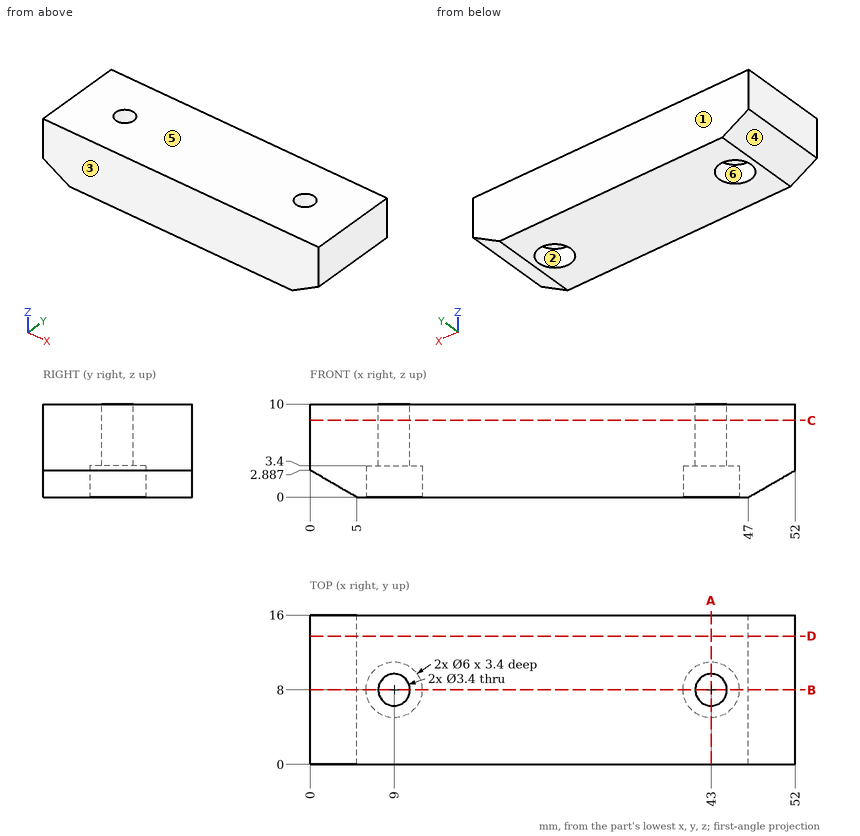
Check sheet for the drawn part. Datum: minimum x, y, z corner. Units: mm. A direction names the side the tool comes from. Give positions to 0.01 mm unless a question says otherwise; leave off trailing zeros. Order: outer loops, then holes, each group sorted by start corner. A loop starts at its lowest first (then second) coordinate and runs counter-clockwise, first axis right, second up. Notation, with made-up numbers: (59.5, 20) - (64.5, 20) arc R19 ccw to (64.5, 48) - close; hole circle Ø2 at (7, 30). An arc over 180 degrees is marked (long way). Answer in a Markdown table with one row per item. Add a question column.
Q1. Mould release check, pull along Y, two halves, no side actions. Record for the marked faces 1, 2, 3 and 4: pulls with the +Y half, pulls with the -Y half, needs draft (parallel to the pull), parting line crosses it, or undercut.
Q2. Tool access check on the marked faces 5 and 6. Record the directions out of +Z, -Z, +X, -X, +Y, -Y that give a thin tool (end or side, any length) a straight path to the whole face; none if there is none.
Q3. Cross-section at B-B, the plane y = 8. Enter the section's corners in (x, z).
Q4. Material ranges on probe 1 along Y at (x, z) = (43, 1.3); probe 2 along Y at (x, z) = (43, 5); probe 3 along X at (y, z) = (6.75, 1.75) (1 decimal), recorded low to high. Write a range as from..to.
Q5. Cross-section at A-A, the plane x = 43. Enter the section's corners in (y, z), then the cut area to 3 significant figures.
Q6. Gauge pin test, flat ends, axial feed: pin 1 (5.5 mm diameter, centred on x = 43, y = 8, fed in from -Z); pin 2 (3 mm diameter, centred on x = 37, z = 7.5, fed in from -Y). Record the tip position at first contact, or that the pin passes through.
Q7. Cross-section at C-C, the plane z = 8.25. Enter the section's corners in (x, y).
Q8. Cross-section at D-D, the plane y = 13.75. Enter the section's corners in (x, z), then the cut area to 3 significant figures.
Check values:
| question | item | result |
|---|---|---|
| 1 | face 1 | pulls with the +Y half |
| 1 | face 2 | undercut |
| 1 | face 3 | pulls with the -Y half |
| 1 | face 4 | needs draft |
| 2 | face 5 | +Z, +X, -X, +Y, -Y |
| 2 | face 6 | -Z |
| 3 | outline | (0, 2.89) - (5, 0) - (6, 0) - (6, 3.4) - (7.3, 3.4) - (7.3, 10) - (0, 10) - close; (10.7, 3.4) - (12, 3.4) - (12, 0) - (40, 0) - (40, 3.4) - (41.3, 3.4) - (41.3, 10) - (10.7, 10) - close; (44.7, 3.4) - (46, 3.4) - (46, 0) - (47, 0) - (52, 2.89) - (52, 10) - (44.7, 10) - close |
| 4 | probe 1 | y = 0..5, 11..16 |
| 4 | probe 2 | y = 0..6.3, 9.7..16 |
| 4 | probe 3 | x = 2..6.3, 11.7..40.3, 45.7..50 |
| 5 | outline | (0, 0) - (5, 0) - (5, 3.4) - (6.3, 3.4) - (6.3, 10) - (0, 10) - close; (9.7, 3.4) - (11, 3.4) - (11, 0) - (16, 0) - (16, 10) - (9.7, 10) - close |
| 5 | area | 117 mm^2 |
| 6 | pin 1 | stops at z = 3.4 |
| 6 | pin 2 | stops at y = 0 |
| 7 | outline | (0, 0) - (52, 0) - (52, 16) - (0, 16) - close; hole circle Ø3.4 at (9, 8); hole circle Ø3.4 at (43, 8) |
| 8 | outline | (0, 2.89) - (5, 0) - (47, 0) - (52, 2.89) - (52, 10) - (0, 10) - close |
| 8 | area | 506 mm^2 |
